from build123d import *

# Parameters (mm, degrees)
BASE_BLOCK_SKETCH_W                = 36
BASE_BLOCK_SKETCH_H                = 24
BASE_BLOCK_DEPTH                   = 36
RECTANGULAR_POCKET_12X6_DEPTH      = 43
RECTANGULAR_POCKET_12X6_DEPTH_BACK = 43
RECTANGULAR_POCKET_SKETCH_W        = 24
RECTANGULAR_POCKET_SKETCH_H        = 12
CLAMP_UPRIGHT_SKETCH_W             = 12
CLAMP_UPRIGHT_SKETCH_H             = 15
CLAMP_UPRIGHT_DEPTH                = 36
CURVED_ARM_DEPTH                   = 15
CLAMP_BLOCK_SKETCH_W               = 30
CLAMP_BLOCK_SKETCH_H               = 15
CLAMP_BLOCK_DEPTH                  = 40
CLAMP_SPLIT_SLOT_1MM_DEPTH         = 101.001249992
CLAMP_SPLIT_SLOT_1MM_DEPTH_BACK    = 101.001249992
CLAMP_CROSS_HOLE_DEPTH             = 111.995495404
CLAMP_CROSS_HOLE_DEPTH_BACK        = 111.995495404
CROSS_HOLE_SKETCH_R                = 3
SIDE_START                         = -18
SIDE_LUG_SKETCH_W                  = 24
SIDE_LUG_SKETCH_H                  = 15
SIDE_LUG_DEPTH                     = 18
ARM_SEGMENT_DEPTH                  = 15
ARM_LINK_DEPTH                     = 15
PIVOT_EYE_SKETCH_R                 = 4.5
PIVOT_EYE_DEPTH                    = 15


with BuildPart() as part:
    # Base Block Sketch → Base Block (new body)
    with BuildSketch(Plane(origin=(0, 0, 0), x_dir=(1, 0, 0), z_dir=(0, 1, 0))):
        Rectangle(BASE_BLOCK_SKETCH_W, BASE_BLOCK_SKETCH_H)
    extrude(amount=BASE_BLOCK_DEPTH)

    # Rectangular Pocket Sketch → Rectangular Pocket 12x6 (cut, two sides: drawn at the far end of the back side and taken through both)
    with BuildSketch(Plane(origin=(0, 36, 0), x_dir=(1, 0, 0), z_dir=(0, 1, 0)).offset(-RECTANGULAR_POCKET_12X6_DEPTH_BACK)):
        Rectangle(RECTANGULAR_POCKET_SKETCH_W, RECTANGULAR_POCKET_SKETCH_H)
    extrude(amount=RECTANGULAR_POCKET_12X6_DEPTH + RECTANGULAR_POCKET_12X6_DEPTH_BACK, mode=Mode.SUBTRACT)

    # Clamp Upright Sketch → Clamp Upright (add)
    with BuildSketch(Plane(origin=(0, 36, 0), x_dir=(1, 0, 0), z_dir=(0, 1, 0))):
        with Locations((24, 0)):
            Rectangle(CLAMP_UPRIGHT_SKETCH_W, CLAMP_UPRIGHT_SKETCH_H)
    extrude(amount=-CLAMP_UPRIGHT_DEPTH)

    # Curved Arm Sketch → Curved Arm (add)
    with BuildSketch(Plane.XY.offset(7.5)):
        with BuildLine():
            Line((30, 36), (62, 36))
            ThreePointArc((62, 36), (52.627416998, 13.372583002), (30, 4))
            Line((30, 4), (30, 36))
        make_face()
    extrude(amount=-CURVED_ARM_DEPTH)

    # Clamp Block Sketch → Clamp Block (add)
    with BuildSketch(Plane(origin=(0, 36, 0), x_dir=(1, 0, 0), z_dir=(0, 1, 0))):
        with Locations((47, 0)):
            Rectangle(CLAMP_BLOCK_SKETCH_W, CLAMP_BLOCK_SKETCH_H)
    extrude(amount=CLAMP_BLOCK_DEPTH)

    # Clamp Split Slot Sketch → Clamp Split Slot 1mm (cut, two sides: drawn at the far end of the back side and taken through both)
    with BuildSketch(Plane.XY.offset(7.5).offset(-CLAMP_SPLIT_SLOT_1MM_DEPTH_BACK)):
        with BuildLine():
            Line((46, 76), (46, 60.94427191))
            ThreePointArc((46, 60.94427191), (47, 43), (48, 60.94427191))
            Line((48, 60.94427191), (48, 76))
            Line((48, 76), (46, 76))
        make_face()
    extrude(amount=CLAMP_SPLIT_SLOT_1MM_DEPTH + CLAMP_SPLIT_SLOT_1MM_DEPTH_BACK, mode=Mode.SUBTRACT)

    # Cross Hole Sketch → Clamp Cross Hole (cut, two sides: drawn at the far end of the back side and taken through both)
    with BuildSketch(Plane(origin=(62, 0, 0), x_dir=(0, 0, -1), z_dir=(1, 0, 0)).offset(-CLAMP_CROSS_HOLE_DEPTH_BACK)):
        with Locations((0, 70)):
            Circle(CROSS_HOLE_SKETCH_R)
    extrude(amount=CLAMP_CROSS_HOLE_DEPTH + CLAMP_CROSS_HOLE_DEPTH_BACK, mode=Mode.SUBTRACT)

    # Side Lug Sketch → Side Lug (add)
    with BuildSketch(Plane(origin=(0, 36, 0), x_dir=(1, 0, 0), z_dir=(0, 1, 0)).offset(SIDE_START)):
        with Locations((-30, -4.5)):
            Rectangle(SIDE_LUG_SKETCH_W, SIDE_LUG_SKETCH_H)
    extrude(amount=-SIDE_LUG_DEPTH)

    # Arm Segment Sketch → Arm Segment (add)
    with BuildSketch(Plane.XY.offset(12)):
        with BuildLine():
            Line((-42, 18), (-42, 28))
            Line((-42, 28), (-60, 28))
            Line((-60, 28), (-60, 18))
            ThreePointArc((-60, 18), (-54.727922061, 5.272077939), (-42, 0))
            Line((-42, 0), (-42, 18))
        make_face()
    extrude(amount=-ARM_SEGMENT_DEPTH)

    # Arm Link Sketch → Arm Link (add)
    with BuildSketch(Plane.XY.offset(12)):
        Polygon((-60, 28), (-42, 28), (-46.393085021, 44), (-64.393085021, 44), align=None)
    extrude(amount=-ARM_LINK_DEPTH)

    # Pivot Eye Sketch → Pivot Eye (add)
    with BuildSketch(Plane.XY.offset(12)):
        with BuildLine():
            Line((-64.393085021, 44), (-64.393085021, 53))
            ThreePointArc((-64.393085021, 53), (-55.393085021, 62), (-46.393085021, 53))
            Line((-46.393085021, 53), (-46.393085021, 44))
            Line((-46.393085021, 44), (-64.393085021, 44))
        make_face()
        with Locations((-55.393085021, 53)):
            Circle(PIVOT_EYE_SKETCH_R, mode=Mode.SUBTRACT)
    extrude(amount=-PIVOT_EYE_DEPTH)


solid = part.part
Could you check a few things on this model? Use its own coordinates, in mm. A direction names the side the tool comes from. Give positions to 0.01 mm unless a question says otherwise; leave off trailing zeros. Order: outer loops, then holes, each group sorted by start corner. A loop starts at its lowest first (then second) coordinate and runs counter-clockwise, first axis right, second up. Notation, with made-up numbers: (53, 68) - (72, 68) arc R6 ccw to (72, 75) - close; hole circle Ø10 at (-8.75, 34.5). An arc over 180 degrees is marked (long way). One line per item, written item: value. Start each with the question number.
1. If I drill on probe 1 along Y at (x, z) = (39.5, 0); probe 2 along X at (y, z) = (52, -3.25); probe 3 along X at (y, z) = (52, 1), over which ranges is the centre line in solid material (lowest first)?
2. Imagine slicing it at C-C on x = 3.5. List the corners of the cut face in (y, z) for me, plus the area to 3 significant figures.
3. For P1, Ø5, axis at x = -15, z = 8.5, coming from the +Y side; P2, Ø11.5, axis at x = -55.39, y = 53, coming from the -Z side; P3, Ø14.5, axis at x = 47, y = 52, coming from the +Z side; P4, Ø7, axis at y = 23.5, z = -5.5, coming from the -X side, each with a flat end and sliding along its axis, tell me the tip position at first contact or that it passes through.
4. For faces 5 (the face through (-30, 18, 4)), 6 (the face through (40, 37, -7.5)), 7 (the face through (-18, 22, -2)), which set-ups out of +Z, -Z, +X, -X, +Y, -Y let a thin tool reach every point of the face, with its end or its side?
5. Thinking about a two-plate mould opening in Z: for faces 1 (the face through (0, 18, 6)), 2 (the face through (0, 18, -12)), 3 (the face through (-60, 23, 5)), 4 (the face through (38.9, 67.07, 0.65)), which applies, +Z half, -Z half, draft (parallel to the pull), parting line (faces both ways), or undercut?
6. Imagine slicing it at A-A on y = 70. List the corners of the cut face in (x, z) for me.
7. Imagine slicing it at D-D on y = 25. List the corners of the cut face in (x, z) for me.
8. Imagine slicing it at B-B on z = 0. Give the number of separate pieces and of enclosed holes in the cut face, plus the area to 3 significant figures.
Values:
1. probe 1: 5.44 to 47.03, 56.97 to 67, 73 to 76
1. probe 2: 32 to 38, 56 to 62
1. probe 3: -64.39 to -59.78, -51.01 to -46.39, 32 to 38, 56 to 62
2. outline: (0, -12) - (36, -12) - (36, -6) - (0, -6) - close; (0, 6) - (36, 6) - (36, 12) - (0, 12) - close
2. area: 432 mm²
3. P1: y = 36
3. P2: z = -3
3. P3: through
3. P4: x = -60
4. face 5: +Z, -Z, +Y
4. face 6: -Z, +X, +Y, -Y
4. face 7: -Z, +Y
5. face 1: undercut
5. face 2: -Z half
5. face 3: draft
5. face 4: undercut
6. outline: (32, -7.5) - (46, -7.5) - (46, -3) - (32, -3) - close; (32, 3) - (46, 3) - (46, 7.5) - (32, 7.5) - close; (48, -7.5) - (62, -7.5) - (62, -3) - (48, -3) - close; (48, 3) - (62, 3) - (62, 7.5) - (48, 7.5) - close
7. outline: (-60, -3) - (-42, -3) - (-42, 12) - (-60, 12) - close; (-18, -12) - (18, -12) - (18, -7.5) - (60.05, -7.5) - (60.05, 7.5) - (18, 7.5) - (18, 12) - (-18, 12) - close; hole (-12, -6) - (12, -6) - (12, 6) - (-12, 6) - close
8. separate pieces: 4
8. enclosed holes: 1
8. area: 3,800 mm²
